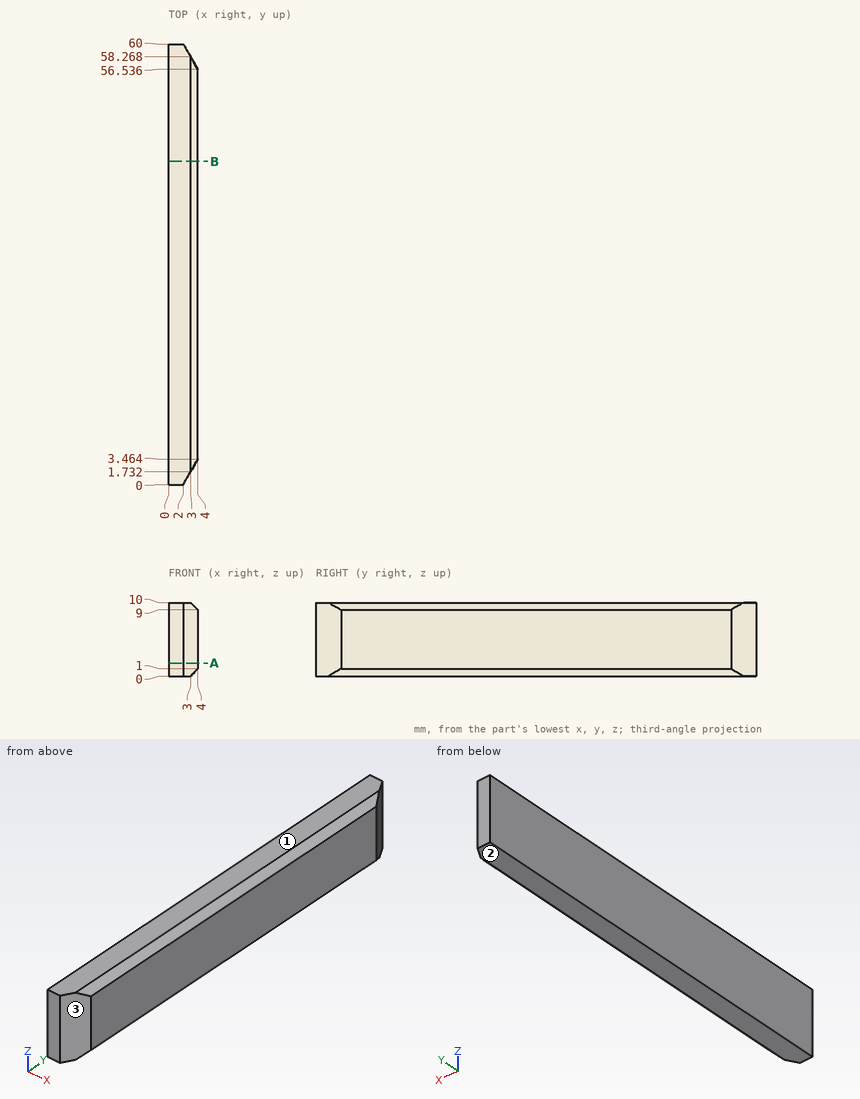
Here's the drawing with two shaded views (mm, measured from the low corner). I have some questions. Round coordinates to 2 decimals unless told otherwise and drop trailing zeros. Loops run counter-clockwise (first coordinate to the right, second up) from the corner with the lowest first, then second, coordinate; pieces in that order, holes last. Notation, with made-up numbers: M -38,70 L 17,70 A19 cw 17,75 Z; hole C 58,-16.75 d5. An arc over 180 degrees is marked long. Answer as a JSON object with one key per item and string values. Group by question number.
Q1. We'd pull the mould along Z, two halves only. Please class the marked faces 1, 2 and 3: +Z half, -Z half, draft (parallel to the pull), parting line (faces both ways), or undercut.
Q2. Imagine slicing it at A-A, the plane z = 1.75. Please give me the cut outline in (x, y), then the cut area to 3 significant figures.
Q3. Imagine slicing it at B-B, the plane y = 44. Please give me the cut outline in (x, z).
Q4. Please list where these lines run through material, in increasing order: L1, parallel to X at y = 3, z = 1; L2, parallel to Y at x = 2.25, z = 7.75; L3, parallel to Z at x = 3.45, y = 10.
Findings:
{
 "1": {"face 1": "+Z half", "face 2": "-Z half", "face 3": "draft"},
 "2": {"outline": "M 0,0 L 2,0 L 4,3.46 L 4,56.54 L 2,60 L 0,60 Z", "area": "233 mm2"},
 "3": {"outline": "M 0,0 L 3,0 L 4,1 L 4,9 L 3,10 L 0,10 Z"},
 "4": {"L1": "x = 0 to 3.73", "L2": "y = 0.43 to 59.57", "L3": "z = 0.45 to 9.55"}
}
